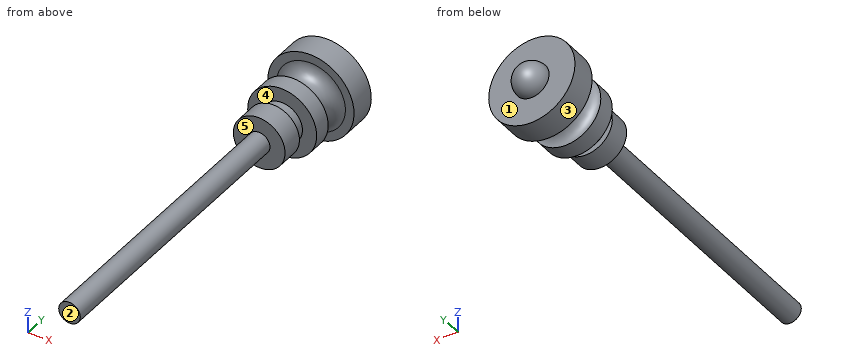
from build123d import *


with BuildPart() as part:
    # Sketch1 → Revolve1 (revolve)
    with BuildSketch(Plane.XY, mode=Mode.PRIVATE) as revolve1_sk:
        Polygon((0, 0), (10, 0), (10, -6), (8, -6), (8, -16), (4.7, -16), (4.7, -19), (6, -19), (6, -24), (2.5, -24), (2.5, -90), (0, -90), align=None)
    revolve(revolve1_sk.sketch.rotate(Axis((0, 0, 0), (0, 1, 0)), 90), axis=Axis((0, 0, 0), (0, 1, 0)))

    # Sketch2 → Cut-Revolve1 (revolve, cut)
    with BuildSketch(Plane.XY, mode=Mode.PRIVATE) as cut_revolve1_sk:
        with BuildLine():
            Line((8, -6), (17.813862568, -6))
            Line((17.813862568, -6), (17.813862568, -12))
            Line((17.813862568, -12), (8, -12))
            ThreePointArc((8, -12), (5, -9), (8, -6))
        make_face()
    revolve(cut_revolve1_sk.sketch.rotate(Axis((0, 5.105729486, 0), (0, -1, 0)), 270), axis=Axis((0, 5.105729486, 0), (0, -1, 0)), mode=Mode.SUBTRACT)

    # Sketch4 → Revolve3 (revolve)
    with BuildSketch(Plane.XY, mode=Mode.PRIVATE) as revolve3_sk:
        with BuildLine():
            Line((0, 4), (0, 0))
            Line((0, 0), (4, 0))
            ThreePointArc((4, 0), (2.828427125, 2.828427125), (0, 4))
        make_face()
    revolve(revolve3_sk.sketch.rotate(Axis((0, 4, 0), (0, -1, 0)), 90), axis=Axis((0, 4, 0), (0, -1, 0)))


solid = part.part
Work out the finished part from the listing and answer in its coordinate system (mm). Face numbers are marked on the shaded views. A direction names the side the tool comes from. Give positions to 0.01 mm unless a question says otherwise; leave off trailing zeros. Loops run counter-clockwise (first coordinate to the right, second up) from the corner with the lowest first, then second, coordinate; pieces in that order, holes last. Notation, with made-up numbers: (-28, -40) -> (18, -40) arc R15 ccw to (18, -36) -> close; hole circle Ø9 at (69.25, 87.25). An arc over 180 degrees is marked (long way). Use a Markdown table: item, result. Add a question column.
1) The part is cut by section A-A, the plane x = 0. Determine the outline of the cut face in (y, z), plus the area to 3 significant figures.
2) Consider line 1 along Y through (x, z) = (7.75, -1); line 2 along Y through (x, z) = (-4.5, 2); line 3 along Y through (x, z) = (2.5, 5). Determine where each line is inside the solid, lowest interval first.
3) Each of these flat-tipped pins is pushed along its axis until it touches: P1, Ø10, axis at y = -45, z = 2, coming from the -X side; P2, Ø5, axis at x = -2.5, z = 5.5, coming from the -Y side; P3, Ø12, axis at x = 7, y = -44, coming from the +Z side; P4, Ø6, axis at x = 2, z = 2.5, coming from the -Y side. Where does it stop, or does it pass through?
4) Which of the six approach directions +Z, -Z, +X, -X, +Y, -Y give full straight-line access (tool end or side, diameter ignored) to the marked faces 1, 2, 3, 4 and 5?
5) The part is cut by section B-B, the plane z = 0. Determine the outline of the cut face in (x, y), plus the area to 3 significant figures.
6) The part is cut by section C-C, the plane y = -75. Determine the outline of the cut face in (x, z), plus the area to 3 significant figures.
Reported:
| question | item | result |
|---|---|---|
| 1 | outline | (-90, -2.5) -> (-24, -2.5) -> (-24, -6) -> (-19, -6) -> (-19, -4.7) -> (-16, -4.7) -> (-16, -8) -> (-12, -8) arc R3 cw to (-6, -8) -> (-6, -10) -> (0, -10) -> (0, -4) arc R4 ccw to (0, 4) -> (0, 10) -> (-6, 10) -> (-6, 8) arc R3 cw to (-12, 8) -> (-16, 8) -> (-16, 4.7) -> (-19, 4.7) -> (-19, 6) -> (-24, 6) -> (-24, 2.5) -> (-90, 2.5) -> close |
| 1 | area | 695 mm^2 |
| 2 | line 1 | y = -16 to -11.99, -6.01 to 0 |
| 2 | line 2 | y = -24 to -19, -16 to 0 |
| 2 | line 3 | y = -24 to -19, -16 to -10.79, -7.21 to 0 |
| 3 | P1 | stops at x = -2.5 |
| 3 | P2 | stops at y = -24 |
| 3 | P3 | stops at z = 2.29 |
| 3 | P4 | stops at y = -90 |
| 4 | face 1 | +Y |
| 4 | face 2 | +Z, -Z, +X, -X, -Y |
| 4 | face 3 | +Y, -Y |
| 4 | face 4 | none |
| 4 | face 5 | -Y |
| 5 | outline | (-10, -6) -> (-8, -6) arc R3 cw to (-8, -12) -> (-8, -16) -> (-4.7, -16) -> (-4.7, -19) -> (-6, -19) -> (-6, -24) -> (-2.5, -24) -> (-2.5, -90) -> (2.5, -90) -> (2.5, -24) -> (6, -24) -> (6, -19) -> (4.7, -19) -> (4.7, -16) -> (8, -16) -> (8, -12) arc R3 cw to (8, -6) -> (10, -6) -> (10, 0) -> (4, 0) arc R4 ccw to (-4, 0) -> (-10, 0) -> close |
| 5 | area | 695 mm^2 |
| 6 | outline | circle Ø5 at (0, 0) |
| 6 | area | 19.6 mm^2 |
